Source: CAD feature listing. Evaluate the final solid. Frame: model axes, mm. Give positions to 0.01 mm unless a question says otherwise; leave off trailing zeros. Order: outer loops, then holes, each group sorted by start corner. A loop starts at its lowest first (then second) coordinate and runs counter-clockwise, first axis right, second up.
from build123d import *

# Parameters (mm, degrees)
SKETCH_1_W          = 363
SKETCH_1_H          = 372
EXTRUDE_1_DEPTH     = 3
SKETCH_2_R          = 15
CUT_EXTRUDE_1_DEPTH = 10
SKETCH_3_W          = 50
SKETCH_3_H          = 90
CUT_EXTRUDE_2_DEPTH = 10
SKETCH_4_W          = 3
SKETCH_4_H          = 192
EXTRUDE_2_DEPTH     = 30
CUT_EXTRUDE_3_DEPTH = 10


with BuildPart() as part:
    # 草图1 → 凸台-拉伸1 (new body)
    with BuildSketch(Plane.XY):
        Rectangle(SKETCH_1_W, SKETCH_1_H)
    extrude(amount=EXTRUDE_1_DEPTH)

    # 草图2 → 切除-拉伸1 (cut)
    with BuildSketch(Plane.XY.offset(3)):
        with Locations((121.5, 136)):
            Circle(SKETCH_2_R)
    extrude(amount=-CUT_EXTRUDE_1_DEPTH, mode=Mode.SUBTRACT)

    # 草图3 → 切除-拉伸2 (cut)
    with BuildSketch(Plane.XY.offset(3)):
        with Locations((-156.5, -141)):
            Rectangle(SKETCH_3_W, SKETCH_3_H)
        with Locations((-156.5, 141)):
            Rectangle(SKETCH_3_W, SKETCH_3_H)
    extrude(amount=-CUT_EXTRUDE_2_DEPTH, mode=Mode.SUBTRACT)

    # 草图4 → 凸台-拉伸2 (add)
    with BuildSketch(Plane.ZY.offset(181.5)):
        with Locations((1.5, 0)):
            Rectangle(SKETCH_4_W, SKETCH_4_H)
    extrude(amount=EXTRUDE_2_DEPTH)

    # 草图5 → 切除-拉伸3 (cut)
    with BuildSketch(Plane.XY.offset(3)):
        with BuildLine():
            Line((165.2, -155.557904139), (165.2, -149.557904139))
            ThreePointArc((165.2, -149.557904139), (168.5, -146.257904139), (171.8, -149.557904139))
            Line((171.8, -149.557904139), (171.8, -155.557904139))
            ThreePointArc((171.8, -155.557904139), (168.5, -158.857904139), (165.2, -155.557904139))
        make_face()
        with BuildLine():
            Line((165.2, 140.283744441), (165.2, 146.283744441))
            ThreePointArc((165.2, 146.283744441), (168.5, 149.583744441), (171.8, 146.283744441))
            Line((171.8, 146.283744441), (171.8, 140.283744441))
            ThreePointArc((171.8, 140.283744441), (168.5, 136.983744441), (165.2, 140.283744441))
        make_face()
        with BuildLine():
            Line((-195.2, 52.919675482), (-195.2, 46.919675482))
            ThreePointArc((-195.2, 46.919675482), (-198.5, 43.619675482), (-201.8, 46.919675482))
            Line((-201.8, 46.919675482), (-201.8, 52.919675482))
            ThreePointArc((-201.8, 52.919675482), (-198.5, 56.219675482), (-195.2, 52.919675482))
        make_face()
        with BuildLine():
            Line((-201.8, -48.714858664), (-201.8, -42.714858664))
            ThreePointArc((-201.8, -42.714858664), (-198.5, -39.414858664), (-195.2, -42.714858664))
            Line((-195.2, -42.714858664), (-195.2, -48.714858664))
            ThreePointArc((-195.2, -48.714858664), (-198.5, -52.014858664), (-201.8, -48.714858664))
        make_face()
    extrude(amount=-CUT_EXTRUDE_3_DEPTH, mode=Mode.SUBTRACT)


solid = part.part
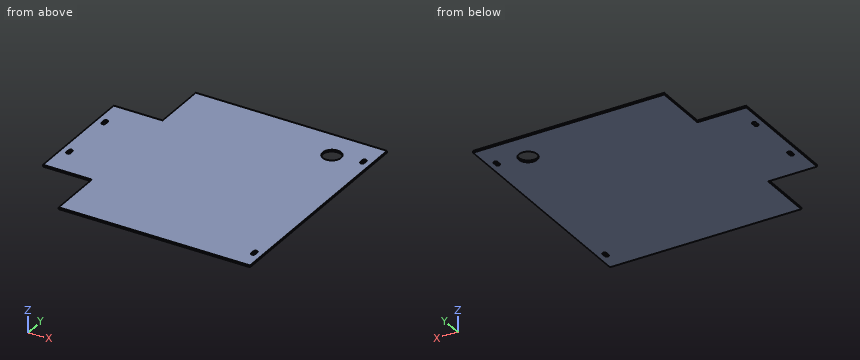
1) Section query B-B on z = 0.55. Output: boundary loops of the cut face in (x, y).
Checks:
outline: (-211.5, -96) - (-131.5, -96) - (-131.5, -186) - (181.5, -186) - (181.5, 186) - (-131.5, 186) - (-131.5, 96) - (-211.5, 96) - close; hole (-201.8, -48.71) arc R3.3 ccw to (-195.2, -48.71) - (-195.2, -42.71) arc R3.3 ccw to (-201.8, -42.71) - close; hole (-201.8, 46.92) arc R3.3 ccw to (-195.2, 46.92) - (-195.2, 52.92) arc R3.3 ccw to (-201.8, 52.92) - close; hole circle Ø30 at (121.5, 136); hole (165.2, -155.56) arc R3.3 ccw to (171.8, -155.56) - (171.8, -149.56) arc R3.3 ccw to (165.2, -149.56) - close; hole (165.2, 140.28) arc R3.3 ccw to (171.8, 140.28) - (171.8, 146.28) arc R3.3 ccw to (165.2, 146.28) - close
2) First-contact query: pin 1 Ø0.9 at (y, z) = (142.5, 1) entering from -X. Flat tip, straight axial feed; report the tip coordinate or a pass-through.
Checks:
pin 1: stops at x = -131.5
3) Section query C-C on y = 101.5. Output: boundary loops of the cut face in (x, z).
Checks:
outline: (-131.5, 0) - (181.5, 0) - (181.5, 3) - (-131.5, 3) - close
4) Ray query, L1, parallel to X at y = 50, z = 1.7; L2, parallel to Y at x = 121.5, z = 2.3; L3, parallel to X at y = -98, z = 1.85. Return the intervals inside material, ascending.
Checks:
L1: x = -211.5 to -201.8, -195.2 to 181.5
L2: y = -186 to 121, 151 to 186
L3: x = -131.5 to 181.5
5) Section query A-A on x = 121.5. Output: boundary loops of the cut face in (y, z).
Checks:
outline: (-186, 0) - (121, 0) - (121, 3) - (-186, 3) - close; (151, 0) - (186, 0) - (186, 3) - (151, 3) - close
